from build123d import *

# Parameters (mm, degrees)
SKETCH1_W              = 100
SKETCH1_H              = 70
SKETCH1_R              = 5.25
BOSS_EXTRUDE1_DEPTH    = 8
SKETCH2_OUTSIDE_W      = 126.466
SKETCH2_OUTSIDE_H      = 96.466
CUT_EXTRUDE1_DEPTH     = 10
M10_TAPPED_HOLE1_D     = 8.5
M10_TAPPED_HOLE1_DEPTH = 24.5
M10_TAPPED_HOLE1_TIP   = 2.553657631


with BuildPart() as part:
    # Sketch1 → Boss-Extrude1 (new body)
    with BuildSketch(Plane.XY.offset(4)):
        with Locations((5.613636364, -1.590909091)):
            Rectangle(SKETCH1_W, SKETCH1_H)
        with Locations(Location((40.613636364, -21.590909091, 0), (0, 0, 180))):
            Circle(SKETCH1_R, mode=Mode.SUBTRACT)
        with Locations(Location((40.613636364, 18.409090909, 0), (0, 0, 180))):
            Circle(SKETCH1_R, mode=Mode.SUBTRACT)
    extrude(amount=-BOSS_EXTRUDE1_DEPTH)

    # Sketch2 outside → Cut-Extrude1 (cut)
    with BuildSketch(Plane.XY.offset(4)):
        with Locations((5.614, -1.591)):
            Rectangle(SKETCH2_OUTSIDE_W, SKETCH2_OUTSIDE_H)
        with BuildLine():
            Line((25.613636364, 33.409090909), (-29.209885446, 23.241423705))
            ThreePointArc((-29.209885446, 23.241423705), (-37.150522341, 15.56807326), (-33.185327877, 5.262188814))
            Line((-33.185327877, 5.262188814), (25.613636364, -36.590909091))
            Line((25.613636364, -36.590909091), (55.613636364, -36.590909091))
            Line((55.613636364, -36.590909091), (55.613636364, 33.409090909))
            Line((55.613636364, 33.409090909), (25.613636364, 33.409090909))
        make_face(mode=Mode.SUBTRACT)
    extrude(amount=-CUT_EXTRUDE1_DEPTH, mode=Mode.SUBTRACT)

    # M10 Tapped Hole1
    with Locations(Plane.XY.offset(4)):
        with Locations((-27.386363636, 13.409090909)):
            Hole(M10_TAPPED_HOLE1_D / 2, depth=M10_TAPPED_HOLE1_DEPTH)
            with Locations((0, 0, -(M10_TAPPED_HOLE1_DEPTH + M10_TAPPED_HOLE1_TIP / 2))):  # 118° drill point
                Cone(0, M10_TAPPED_HOLE1_D / 2, M10_TAPPED_HOLE1_TIP, mode=Mode.SUBTRACT)


solid = part.part
Geometry: final body of the model. Coordinates: model frame, mm. Round coordinates to 2 decimals unless told otherwise and drop trailing zeros. Order: outer loops, then holes, each group sorted by start corner. A loop starts at its lowest first (then second) coordinate and runs counter-clockwise, first axis right, second up.
Q1. Section C-C, the plane z = -0.25. Output: boundary loops of the cut face in (x, y).
Result sheet:
outline: (-33.19, 5.26) - (25.61, -36.59) - (55.61, -36.59) - (55.61, 33.41) - (25.61, 33.41) - (-29.21, 23.24) arc R10 ccw to start; hole circle Ø8.5 at (-27.39, 13.41); hole circle Ø10.5 at (40.61, -21.59); hole circle Ø10.5 at (40.61, 18.41)
Q2. Material intervals for probe 1 along X at (y, z) = (14, -0.25); probe 2 along Y at (x, z) = (43, -3.5); probe 3 along Y at (x, z) = (-31, 3), sorted ascending.
Result sheet:
probe 1: x = -37.37 to -31.6, -23.18 to 37.76, 43.46 to 55.61
probe 2: y = -36.59 to -26.27, -16.91 to 13.73, 23.09 to 33.41
probe 3: y = 3.71 to 11.17, 15.65 to 22.73
Q3. Section D-D, the plane y = -11.5. Output: boundary loops of the cut face in (x, z).
Result sheet:
outline: (-9.64, -4) - (55.61, -4) - (55.61, 4) - (-9.64, 4) - close
Q4. Section B-B, the plane x = -25. Output: boundary loops of the cut face in (y, z).
Result sheet:
outline: (-0.56, -4) - (9.89, -4) - (9.89, 4) - (-0.56, 4) - close; (16.93, -4) - (24.02, -4) - (24.02, 4) - (16.93, 4) - close
Q5. Section A-A, the plane y = 19.5. Output: boundary loops of the cut face in (x, z), and give its area (3 significant figures).
Result sheet:
outline: (-35.32, -4) - (35.48, -4) - (35.48, 4) - (-35.32, 4) - close; (45.75, -4) - (55.61, -4) - (55.61, 4) - (45.75, 4) - close
area: 645 mm2
Q6. Mould query, pull axis Y, two halves, no side actions, for faces 1 (the face through (-1.4, 28.4, 0.1)), 2 (the face through (19, 7, -4)), 3 (the face through (35.606, -23.168, 0.056)). Classes: released by +Y, released by -Y, zero draft, split by the parting line, or undercut.
Result sheet:
face 1: released by +Y
face 2: zero draft
face 3: undercut
Q7. Pin query (flat end, axial travel): pin 1 (2 mm diameter, centred on y = 14.5, z = -2.5, fed in from -X); pin 2 (1 mm diameter, centred on x = -2.5, z = 1.5, fed in from -Y); pin 3 (9.5 mm diameter, centred on x = 40.61, y = 18.41, fed in from -Z) (1 decimal); pin 4 (1 mm diameter, centred on x = 22, z = 2.5, fed in from -Y). Return the tip coordinate at first contact, or that it passes through.
Result sheet:
pin 1: stops at x = -37.39
pin 2: stops at y = -16.94
pin 3: passes through
pin 4: stops at y = -34.37
